CAD build for the part. Positions are in the model's coordinates, mm. A direction names the side the tool comes from. Coordinates: 2 decimals unless noted, no trailing zeros. Order: outer loops, then holes, each group sorted by start corner. A loop starts at its lowest first (then second) coordinate and runs counter-clockwise, first axis right, second up. Notation, with made-up numbers: (43.5, -25.5) - (65.5, -25.5) arc R20 ccw to (65.5, 10.5) - close; hole circle Ø6 at (82.25, -21.5). An arc over 180 degrees is marked (long way). Return JSON: item names as keys, results as strings.
from build123d import *

# Parameters (mm, degrees)
EXTRUDE_1_DEPTH     = 165
SKETCH_3_R          = 20
CUT_EXTRUDE_1_DEPTH = 25


with BuildPart() as part:
    # 草图2 → 拉伸-薄壁1 (new, symmetric)
    with BuildSketch(Plane.XY):
        with BuildLine():
            Line((-12.3, 15), (12.3, 15))
            ThreePointArc((12.3, 15), (14.209188309, 14.209188309), (15, 12.3))
            Line((15, 12.3), (15, -12.3))
            ThreePointArc((15, -12.3), (14.209188309, -14.209188309), (12.3, -15))
            Line((12.3, -15), (-12.3, -15))
            ThreePointArc((-12.3, -15), (-14.209188309, -14.209188309), (-15, -12.3))
            Line((-15, -12.3), (-15, 12.3))
            ThreePointArc((-15, 12.3), (-14.209188309, 14.209188309), (-12.3, 15))
        make_face()
        with BuildLine():
            Line((-12.3, 12.5), (12.3, 12.5))
            ThreePointArc((12.3, 12.5), (12.441421356, 12.441421356), (12.5, 12.3))
            Line((12.5, 12.3), (12.5, -12.3))
            ThreePointArc((12.5, -12.3), (12.441421356, -12.441421356), (12.3, -12.5))
            Line((12.3, -12.5), (-12.3, -12.5))
            ThreePointArc((-12.3, -12.5), (-12.441421356, -12.441421356), (-12.5, -12.3))
            Line((-12.5, -12.3), (-12.5, 12.3))
            ThreePointArc((-12.5, 12.3), (-12.441421356, 12.441421356), (-12.3, 12.5))
        make_face(mode=Mode.SUBTRACT)
    extrude(amount=EXTRUDE_1_DEPTH, both=True)

    # 草图3 → 切除-拉伸1 (cut, symmetric)
    with BuildSketch(Plane(origin=(0, 0, 0), x_dir=(1, 0, 0), z_dir=(0, 1, 0))):
        with Locations((0, -165)):
            Circle(SKETCH_3_R)
        with Locations((0, 165)):
            Circle(SKETCH_3_R)
    extrude(amount=CUT_EXTRUDE_1_DEPTH, both=True, mode=Mode.SUBTRACT)


solid = part.part
Item 1: Mould opens along Y. For faces 1 (the flat face through (0, -15, 2)), 2 (the flat face through (-12.5, 0, 2)), 3 (the flat face through (0, 12.5, 2)), 4 (the flat face through (-15, 0, 2)) say: released by +Y, released by -Y, zero draft, split by the parting line, or undercut.
Findings below:
{"face 1": "released by -Y", "face 2": "undercut", "face 3": "undercut", "face 4": "zero draft"}
Item 2: Band-saw the part on A-A, the plane y = 5. List the corners of the cut face in (x, z).
Findings below:
{"outline": "(-15, -151.77) arc R20 cw to (-12.5, -149.39) - (-12.5, 149.39) arc R20 cw to (-15, 151.77) - close; (12.5, -149.39) arc R20 cw to (15, -151.77) - (15, 151.77) arc R20 cw to (12.5, 149.39) - close"}
Item 3: Wall check: L1, parallel to X at y = 6, z = 30; L2, parallel to X at y = 13.5, z = 95. Give the ranges that are in metal, low to high. Write a range as [from, to].
Findings below:
{"L1": "x = [-15, -12.5], [12.5, 15]", "L2": "x = [-14.72, 14.72]"}
Item 4: Band-saw the part on C-C, the plane z = -100.5. List the corners of the cut face in (x, y).
Findings below:
{"outline": "(-15, -12.3) arc R2.7 ccw to (-12.3, -15) - (12.3, -15) arc R2.7 ccw to (15, -12.3) - (15, 12.3) arc R2.7 ccw to (12.3, 15) - (-12.3, 15) arc R2.7 ccw to (-15, 12.3) - close; hole (-12.5, -12.3) arc R0.2 ccw to (-12.3, -12.5) - (12.3, -12.5) arc R0.2 ccw to (12.5, -12.3) - (12.5, 12.3) arc R0.2 ccw to (12.3, 12.5) - (-12.3, 12.5) arc R0.2 ccw to (-12.5, 12.3) - close"}
Item 5: Band-saw the part on B-B, the plane x = 3. List the corners of the cut face in (y, z), then the cut area to 3 significant figures.
Findings below:
{"outline": "(-15, -145.23) - (-12.5, -145.23) - (-12.5, 145.23) - (-15, 145.23) - close; (12.5, -145.23) - (15, -145.23) - (15, 145.23) - (12.5, 145.23) - close", "area": "1,450 mm²"}
Item 6: Drop a flat-ended pin along its axis: P1, Ø8, axis at x = 10, y = -10.5, coming from the -Z side. Give the stop position or say it passes through.
Findings below:
{"P1": "stops at z = -150.72"}
Item 7: Which spindle directions (+Z, -Z, +X, -X, +Y, -Y) get a long thin tool onto all of the face, cutting with end or side? Do faces 5 (the cylindrical face through (-13.86, 0.21, -150.58)), 6 (the flat face through (12.5, 0, 2)). Say none if no direction does.
Findings below:
{"face 5": "-Z, +Y, -Y", "face 6": "+Z, -Z"}
